For this review, take the finished solid that the model builds, in its own axes (mm). Face numbers are marked on the shaded views. A direction names the side the tool comes from. Give positions to 0.01 mm unless a question says otherwise; leave off trailing zeros. Loops run counter-clockwise (first coordinate to the right, second up) from the corner with the lowest first, then second, coordinate; pieces in that order, holes last.
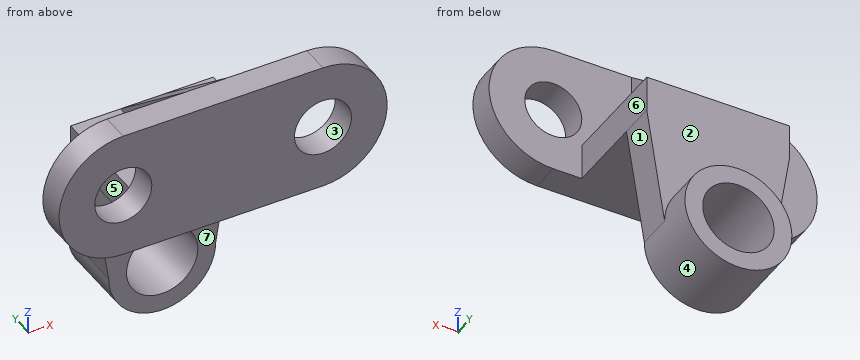
```python
from build123d import *

# Parameters (mm, degrees)
BASE_PLATE_SKETCH_W        = 92
BASE_PLATE_SKETCH_H        = 36
BASE_PLATE_DEPTH           = 8
BASE_PLATE_FILLET_A_RADIUS = 18
BASE_PLATE_FILLET_A_LENGTH = 8
BASE_PLATE_FILLET_B_RADIUS = 18
BASE_PLATE_FILLET_B_LENGTH = 8
MOUNTING_HOLES_SKETCH_R    = 8
MOUNTING_HOLES_2X_DEPTH    = 51.039984013
PEDESTAL_SKETCH_W          = 40
PEDESTAL_SKETCH_H          = 32
CENTRAL_PEDESTAL_DEPTH     = 10
GUSSET_RIB_DEPTH           = 12
UPPER_ARM_DEPTH            = 10
HUB_START                  = 10
HUB_BOSS_SKETCH_R          = 15
HUB_BOSS_SKETCH_R_2        = 10
HUB_BOSS_DEPTH             = 10
HUB_BORE_SKETCH_R          = 10
HUB_BORE_DEPTH             = 90.112288715


with BuildPart() as part:
    # Base Plate Sketch → Base Plate (new body)
    with BuildSketch(Plane(origin=(0, 0, 0), x_dir=(1, 0, 0), z_dir=(0, 1, 0))):
        Rectangle(BASE_PLATE_SKETCH_W, BASE_PLATE_SKETCH_H)
    extrude(amount=BASE_PLATE_DEPTH)

    # Base Plate Fillet A: full round fillet: the end face becomes a half cylinder, R = half its width
    base_plate_fillet_a_face = Plane((46, 4, 0), x_dir=(0, -1, 0), z_dir=(1, 0, 0))  # on the end face: x along it, z out of the body
    base_plate_fillet_a_slab = base_plate_fillet_a_face.offset(-BASE_PLATE_FILLET_A_RADIUS / 2) * Box(BASE_PLATE_FILLET_A_LENGTH, 2 * BASE_PLATE_FILLET_A_RADIUS, BASE_PLATE_FILLET_A_RADIUS, mode=Mode.PRIVATE)  # the body's end, R deep
    base_plate_fillet_a_round = Plane((28, 4, 0), x_dir=(1, 0, 0), z_dir=(0, -1, 0)) * Cylinder(BASE_PLATE_FILLET_A_RADIUS, BASE_PLATE_FILLET_A_LENGTH, mode=Mode.PRIVATE)  # its axis R under the face
    add(base_plate_fillet_a_slab - base_plate_fillet_a_round, mode=Mode.SUBTRACT)

    # Base Plate Fillet B: full round fillet: the end face becomes a half cylinder, R = half its width
    base_plate_fillet_b_face = Plane((-46, 4, 0), x_dir=(0, 1, 0), z_dir=(-1, 0, 0))  # on the end face: x along it, z out of the body
    base_plate_fillet_b_slab = base_plate_fillet_b_face.offset(-BASE_PLATE_FILLET_B_RADIUS / 2) * Box(BASE_PLATE_FILLET_B_LENGTH, 2 * BASE_PLATE_FILLET_B_RADIUS, BASE_PLATE_FILLET_B_RADIUS, mode=Mode.PRIVATE)  # the body's end, R deep
    base_plate_fillet_b_round = Plane((-28, 4, 0), x_dir=(-1, 0, 0), z_dir=(0, 1, 0)) * Cylinder(BASE_PLATE_FILLET_B_RADIUS, BASE_PLATE_FILLET_B_LENGTH, mode=Mode.PRIVATE)  # its axis R under the face
    add(base_plate_fillet_b_slab - base_plate_fillet_b_round, mode=Mode.SUBTRACT)

    # Mounting Holes Sketch → Mounting Holes 2x (cut, through all)
    with BuildSketch(Plane(origin=(0, 8, 0), x_dir=(1, 0, 0), z_dir=(0, 1, 0))):
        with Locations(Location((-28, 0, 0), (0, 0, 270))):
            Circle(MOUNTING_HOLES_SKETCH_R)
        with Locations(Location((28, 0, 0), (0, 0, 270))):
            Circle(MOUNTING_HOLES_SKETCH_R)
    extrude(amount=-MOUNTING_HOLES_2X_DEPTH, mode=Mode.SUBTRACT)

    # Pedestal Sketch → Central Pedestal (add)
    with BuildSketch(Plane(origin=(0, 0, -18), x_dir=(-1, 0, 0), z_dir=(0, 0, -1))):
        with Locations((0, 24)):
            Rectangle(PEDESTAL_SKETCH_W, PEDESTAL_SKETCH_H)
    extrude(amount=-CENTRAL_PEDESTAL_DEPTH)

    # Gusset Rib Sketch → Gusset Rib (add)
    with BuildSketch(Plane(origin=(-6, 0, 0), x_dir=(0, 0, -1), z_dir=(1, 0, 0))):
        Polygon((8, 40), (-18, 8), (8, 8), align=None)
    extrude(amount=GUSSET_RIB_DEPTH)

    # Upper Arm Sketch → Upper Arm (add)
    with BuildSketch(Plane(origin=(0, 40, 0), x_dir=(1, 0, 0), z_dir=(0, 1, 0))):
        with BuildLine():
            Line((-20, 18), (20, 18))
            Line((20, 18), (15, 50))
            ThreePointArc((15, 50), (0, 65), (-15, 50))
            Line((-15, 50), (-20, 18))
        make_face()
    extrude(amount=-UPPER_ARM_DEPTH)

    # Hub Boss Sketch → Hub Boss (add)
    with BuildSketch(Plane(origin=(0, 40, 0), x_dir=(1, 0, 0), z_dir=(0, 1, 0)).offset(HUB_START)):
        with Locations(Location((0, 50, 0), (0, 0, 270))):
            Circle(HUB_BOSS_SKETCH_R)
        with Locations(Location((0, 50, 0), (0, 0, 270))):
            Circle(HUB_BOSS_SKETCH_R_2, mode=Mode.SUBTRACT)
    extrude(amount=-HUB_BOSS_DEPTH)

    # Hub Bore Sketch → Hub Bore (cut, through all)
    with BuildSketch(Plane(origin=(0, 40, 0), x_dir=(1, 0, 0), z_dir=(0, 1, 0))):
        with Locations(Location((0, 50, 0), (0, 0, 270))):
            Circle(HUB_BORE_SKETCH_R)
    extrude(amount=-HUB_BORE_DEPTH, mode=Mode.SUBTRACT)


solid = part.part
```
Q1. Consider section D-D on x = 16.5. Give the boundary of the cut face in (y, z).
Answers:
outline: (0, -18) - (30, -18) - (30, -40.4) - (40, -40.4) - (40, -8) - (8, -8) - (8, 18) - (0, 18) - close
Q2. Consider section A-A on x = 0. Give the boundary of the cut face in (y, z), plus the area to 3 significant figures.
Answers:
outline: (0, -18) - (30, -18) - (30, -40) - (50, -40) - (50, -35) - (40, -35) - (40, -8) - (8, 18) - (0, 18) - close; (30, -65) - (50, -65) - (50, -60) - (30, -60) - close
area: 1,390 mm2
Q3. Machinability: for the marked faces 4, 5, 6 and 7, which of the approach directions +Z, -Z, +X, -X, +Y, -Y give a long, thin tool a straight path to every point of the face, cutting with its end or side? Answer none if there is none.
Answers:
face 4: +Y
face 5: +Z, -Z, -X, +Y
face 6: +Z, -Z, +X, +Y
face 7: -Z, +X, -X, -Y
Q4. Mouldability with a two-part tool opening along Z and no side actions: class the marked faces 1, 2 and 3 as +Z half, -Z half, draft (parallel to the pull), parting line (faces both ways), or undercut.
Answers:
face 1: -Z half
face 2: draft
face 3: undercut
Q5. For pin 1 Ø21 at (y, z) = (16, 4.5) entering from +X; pin 2 Ø8 at (y, z) = (20, -12.5) entering from +X; pin 3 Ø13 at (y, z) = (21.5, 3.5) entering from -X; pin 4 Ø14.5 at (x, z) = (28, 0) entering from -Y, all flat-tipped, find the tip position at first contact; note any pin that passes through.
Answers:
pin 1: stops at x = 46
pin 2: stops at x = 20
pin 3: stops at x = -6
pin 4: passes through
Q6. Consider section C-C on z = -44. Give the boundary of the cut face in (x, y).
Answers:
outline: (-15.94, 30) - (-8, 30) - (-8, 50) - (-13.75, 50) - (-13.75, 40) - (-15.94, 40) - close; (8, 30) - (15.94, 30) - (15.94, 40) - (13.75, 40) - (13.75, 50) - (8, 50) - close
Q7. Consider section B-B on y = 16. Give the boundary of the cut face in (x, z), plus the area to 3 significant figures.
Answers:
outline: (-20, -18) - (20, -18) - (20, -8) - (6, -8) - (6, 11.5) - (-6, 11.5) - (-6, -8) - (-20, -8) - close
area: 634 mm2
Q8. For probe 1 along X at (y, z) = (4.5, 0); probe 2 along X at (y, z) = (36.25, -50); probe 3 along Z at (x, y) = (12, 15), list the stretches that pass through material, from the lowest coordinate up.
Answers:
probe 1: x = -46 to -36, -20 to 20, 36 to 46
probe 2: x = -15 to -10, 10 to 15
probe 3: z = -18 to -8
